Build history of the part. All positions in model axes, mm. Face numbers are marked on the shaded views. A direction names the side the tool comes from. Round coordinates to 2 decimals unless told otherwise and drop trailing zeros. Write each loop counter-clockwise with the first axis right and the second up, starting at its lowest first coordinate (ties: lowest second). Pieces come first, ordered by that corner, then holes.
from build123d import *

# Parameters (mm, degrees)
BASE_BLOCK_SKETCH_W         = 110
BASE_BLOCK_SKETCH_H         = 20
BASE_BLOCK_DEPTH            = 60
BEARING_SADDLE_64_DEPTH     = 64
SADDLE_BORE_36_DEPTH        = 84
LEFT_MOUNTING_LUG_DEPTH     = 22
LEFT_LUG_HOLE_SKETCH_R      = 6
LEFT_LUG_HOLE_12_DEPTH      = 22
RIGHT_MOUNTING_LUG_DEPTH    = 22
RIGHT_LUG_HOLE_SKETCH_R     = 6
RIGHT_LUG_HOLE_12_DEPTH     = 22
UPRIGHT_PLATE_DEPTH         = 10
UPRIGHT_PLATE_DEPTH_BACK    = 30
UPRIGHT_PLATE_SKETCH_R      = 22
UPRIGHT_REINFORCEMENT_DEPTH = 10
UPPER_BORE_SKETCH_R         = 11
UPPER_BORE_22_DEPTH         = 40
GUSSET_BOSS_DEPTH           = 64
GUSSET_RELIEF_CUT_DEPTH     = 64
GUSSET_TRIM_CUT_DEPTH       = 10
UPRIGHT_HOLE_A_SKETCH_R     = 7.5
UPRIGHT_HOLE_A_15_DEPTH     = 20
UPRIGHT_HOLE_B_SKETCH_R     = 7.5
UPRIGHT_HOLE_B_15_DEPTH     = 20


with BuildPart() as part:
    # Base Block Sketch → Base Block (new body)
    with BuildSketch(Plane(origin=(0, 0, 0), x_dir=(1, 0, 0), z_dir=(0, 1, 0))):
        with Locations((0, 10)):
            Rectangle(BASE_BLOCK_SKETCH_W, BASE_BLOCK_SKETCH_H)
    extrude(amount=BASE_BLOCK_DEPTH)

    # Bearing Saddle Sketch → Bearing Saddle Ø64 (add)
    with BuildSketch(Plane.XY):
        with BuildLine():
            Line((-32, 0), (32, 0))
            ThreePointArc((32, 0), (0, 32), (-32, 0))
        make_face()
    extrude(amount=BEARING_SADDLE_64_DEPTH)

    # Saddle Bore Sketch → Saddle Bore Ø36 (cut)
    with BuildSketch(Plane.XY.offset(64)):
        with BuildLine():
            Line((-18, 0), (18, 0))
            ThreePointArc((18, 0), (0, 18), (-18, 0))
        make_face()
    extrude(amount=-SADDLE_BORE_36_DEPTH, mode=Mode.SUBTRACT)

    # Left Lug Sketch → Left Mounting Lug (add)
    with BuildSketch(Plane(origin=(0, 0, 0), x_dir=(1, 0, 0), z_dir=(0, 1, 0))):
        with BuildLine():
            Line((-40, -17), (-18.724275485, -17))
            Line((-18.724275485, -17), (-18.724275485, -47))
            Line((-18.724275485, -47), (-40, -47))
            ThreePointArc((-40, -47), (-55, -32), (-40, -17))
        make_face()
    extrude(amount=LEFT_MOUNTING_LUG_DEPTH)

    # Left Lug Hole Sketch → Left Lug Hole Ø12 (cut)
    with BuildSketch(Plane(origin=(0, 22, 0), x_dir=(1, 0, 0), z_dir=(0, 1, 0))):
        with Locations(Location((-40, -32, 0), (0, 0, 270))):
            Circle(LEFT_LUG_HOLE_SKETCH_R)
    extrude(amount=-LEFT_LUG_HOLE_12_DEPTH, mode=Mode.SUBTRACT)

    # Right Lug Sketch → Right Mounting Lug (add)
    with BuildSketch(Plane(origin=(0, 0, 0), x_dir=(1, 0, 0), z_dir=(0, 1, 0))):
        with BuildLine():
            Line((40, -17), (17.182133471, -17))
            Line((17.182133471, -17), (17.182133471, -47))
            Line((17.182133471, -47), (39.293701119, -46.983362169))
            ThreePointArc((39.293701119, -46.983362169), (54.995839965, -32.353247409), (40, -17))
        make_face()
    extrude(amount=RIGHT_MOUNTING_LUG_DEPTH)

    # Right Lug Hole Sketch → Right Lug Hole Ø12 (cut)
    with BuildSketch(Plane(origin=(0, 22, 0), x_dir=(1, 0, 0), z_dir=(0, 1, 0))):
        with Locations(Location((40, -32, 0), (0, 0, 270))):
            Circle(RIGHT_LUG_HOLE_SKETCH_R)
    extrude(amount=-RIGHT_LUG_HOLE_12_DEPTH, mode=Mode.SUBTRACT)



with BuildPart() as body_2:
    # Upright Plate Sketch → Upright Plate (new, two sides: drawn at the far end of the back side and taken through both)
    with BuildSketch(Plane.XY.offset(-UPRIGHT_PLATE_DEPTH_BACK)):
        with Locations((0, 100)):
            Circle(UPRIGHT_PLATE_SKETCH_R)
    extrude(amount=UPRIGHT_PLATE_DEPTH + UPRIGHT_PLATE_DEPTH_BACK)


with BuildPart() as part_1:
    add(part.part)

    add(body_2.part)  # Upright Reinforcement merges body 2
    # Upright Reinforcement Sketch → Upright Reinforcement (add)
    with BuildSketch(Plane.XY):
        with BuildLine():
            Line((-55, 60), (-17.999682143, 112.649562947))
            ThreePointArc((-17.999682143, 112.649562947), (0, 78), (17.999682143, 112.649562947))
            Line((17.999682143, 112.649562947), (55, 60))
            Line((55, 60), (-55, 60))
        make_face()
    extrude(amount=-UPRIGHT_REINFORCEMENT_DEPTH)

    # Upper Bore Sketch → Upper Bore Ø22 (cut)
    with BuildSketch(Plane.XY.offset(10)):
        with Locations((0, 100)):
            Circle(UPPER_BORE_SKETCH_R)
    extrude(amount=-UPPER_BORE_22_DEPTH, mode=Mode.SUBTRACT)

    # Gusset Boss Sketch → Gusset Boss (add)
    with BuildSketch(Plane.XY):
        with BuildLine():
            Line((-5, 78.575714714), (-5, 31.606961259))
            ThreePointArc((-5, 31.606961259), (0, 32), (5, 31.606961259))
            Line((5, 31.606961259), (5, 78.575714714))
            ThreePointArc((5, 78.575714714), (0, 78), (-5, 78.575714714))
        make_face()
    extrude(amount=GUSSET_BOSS_DEPTH)

    # Gusset Relief Sketch → Gusset Relief Cut (cut)
    with BuildSketch(Plane(origin=(0, 0, 0), x_dir=(0, 0, -1), z_dir=(1, 0, 0))):
        Polygon((-10, 78.575714714), (-64, 31.606961259), (-64, 78.575714714), align=None)
    extrude(amount=-GUSSET_RELIEF_CUT_DEPTH, mode=Mode.SUBTRACT)

    # Gusset Trim Sketch → Gusset Trim Cut (cut)
    with BuildSketch(Plane.ZY):
        Polygon((10, 78.575714714), (64, 31.606961259), (64, 78.575714714), align=None)
    extrude(amount=-GUSSET_TRIM_CUT_DEPTH, mode=Mode.SUBTRACT)

    # Upright Hole A Sketch → Upright Hole A Ø15 (cut)
    with BuildSketch(Plane.XY):
        with Locations((40, 44)):
            Circle(UPRIGHT_HOLE_A_SKETCH_R)
    extrude(amount=-UPRIGHT_HOLE_A_15_DEPTH, mode=Mode.SUBTRACT)

    # Upright Hole B Sketch → Upright Hole B Ø15 (cut)
    with BuildSketch(Plane.XY):
        with Locations((-40, 44)):
            Circle(UPRIGHT_HOLE_B_SKETCH_R)
    extrude(amount=-UPRIGHT_HOLE_B_15_DEPTH, mode=Mode.SUBTRACT)


solid = part_1.part
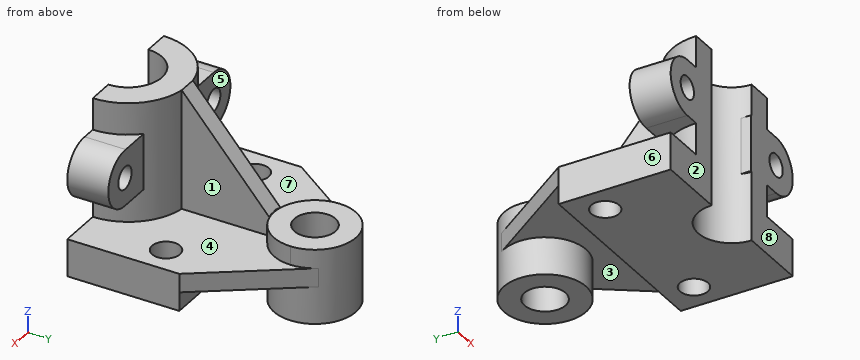
1) Which spindle directions (+Z, -Z, +X, -X, +Y, -Y) get a long thin tool onto all of the face, cutting with end or side? Do the marked faces 1, 2, 3, 4 and 5. Say none if no direction does.
Results:
face 1: +Z, +X
face 2: +Z, -Z, +X, -X, -Y
face 3: -Z
face 4: +X
face 5: +Z, -X, +Y
2) Slice it at B-B (x = -8). Write the cut outline in (y, z).
Results:
outline: (16.12, -20) - (60, -20) - (60, -10) - (79.51, -10) - (79.51, -30) - (92.45, -30) - (92.45, 10) - (79.51, 10) - (79.51, 0) - (30.98, 0) - (30.98, 64) - (16.12, 64) - close; (107.55, -30) - (120.49, -30) - (120.49, 10) - (107.55, 10) - close
3) Slice it at A-A (z = -6). Write the cut outline in (x, y), plus the area to 3 significant figures.
Results:
outline: (-55, 0) - (-18, 0) arc R18 cw to (18, 0) - (55, 0) - (55, 60) - (18, 112.65) arc R22 ccw to (-18, 112.65) - (-55, 60) - close; hole circle Ø15 at (-40, 44); hole circle Ø22 at (0, 100); hole circle Ø15 at (40, 44)
area: 9,440 mm2
4) Mould opens along Y. For the marked faces 6, 7 and 8 say: released by +Y, released by -Y, zero draft, split by the parting line, or undercut.
Results:
face 6: zero draft
face 7: undercut
face 8: released by -Y
5) Slice it at D-D (z = 32). Write the cut outline in (x, y).
Results:
outline: (-55, 0) - (-46, 0) - (-46, 22) - (-55, 22) - close; (-34, 0) - (-18, 0) arc R18 cw to (17.18, 5.36) - (17.18, 0) - (34, 0) - (34, 22) - (23.24, 22) arc R32 ccw to (5, 31.61) - (5, 59.44) - (-5, 59.44) - (-5, 31.61) arc R32 ccw to (-23.24, 22) - (-34, 22) - close; (46, 0) - (55, 0) - (55, 22) - (46, 22) - close
6) Slice it at C-C (y = 12.5). Write the cut outline in (x, z).
Results:
outline: (-55, -20) - (-12.95, -20) - (-12.95, 64) - (-29.46, 64) - (-29.46, 47) - (-40, 47) arc R15 ccw to (-40, 17) - (-29.46, 17) - (-29.46, 0) - (-55, 0) - close; (12.95, -20) - (55, -20) - (55, 0) - (29.46, 0) - (29.46, 17) - (40, 17) arc R15 ccw (long way) to (39.29, 46.98) - (29.46, 46.99) - (29.46, 64) - (12.95, 64) - close; hole circle Ø12 at (-40, 32); hole circle Ø12 at (40, 32)
7) Pin check, flat tips, straight feed: pin 1 Ø0.9 at (x, y) = (17.5, 4) entering from -Z; pin 2 Ø12 at (y, z) = (108.5, 14.5) entering from -X; pin 3 Ø17 at (x, y) = (-40, 44) entering from +Z; pin 4 Ø5 at (y, z) = (69.5, 25.5) entering from -X. Stop position of each tip, or through.
Results:
pin 1: stops at z = -20
pin 2: stops at x = -21.53
pin 3: stops at z = 0
pin 4: passes through
8) Wall check: L1, parallel to Y at x = 0, z = -19; L2, parallel to Z at x = -33.5, y = 69; L3, parallel to X at y = 39.5, z = 30. Give the ranges that are in metal, low to high.
Results:
L1: y = 18 to 60, 78 to 89, 111 to 122
L2: z = -10 to 0
L3: x = -5 to 5
